Input: part model. Units: mm. Frame: model coordinates. Face numbers are marked on the shaded views. A direction names the side the tool comes from. Give positions to 0.01 mm unless a question says otherwise; leave off trailing zeros. Write each loop counter-clockwise with the first axis right and the second up, starting at its lowest first coordinate (ties: lowest second). Pieces come first, ordered by that corner, then holes. Notation, with made-up numbers: (82, 61) - (89, 61) arc R14 ccw to (89, 83) - close; hole circle Ø10 at (6, 85.25). An arc over 180 degrees is marked (long way). Use a Markdown table: item, result. Add a question column.
1. Section query D-D, the plane y = 53. Return loops of the section in (x, z).
2. Section query B-B, the plane z = -82.5. Return loops of the section in (x, y), plus the area to 3 significant figures.
3. Section query C-C, the plane x = 6.5. Return loops of the section in (y, z).
4. Set-up query: the marked faces 1, 2, 3, 4 and 5. Return all of +Z, -Z, +X, -X, +Y, -Y with unobstructed straight access to the full face (end or side cutting, diameter ignored); none if empty.
5. Material intervals for probe 1 along X at (y, z) = (-10, -135); probe 2 along Z at (x, y) = (19, -50); probe 3 along X at (y, z) = (86, -74.5), sorted ascending.
6. Section query A-A, the plane x = 39. Return loops of the section in (y, z), plus the area to 3 significant figures.
7. Pin query (flat end, axial travel): pin 1 (12 mm diameter, centred on x = 1.5, z = -126, fed in from +Y); pin 2 (2 mm diameter, centred on x = -46.5, y = 85, fed in from -Z); pin 3 (4 mm diameter, centred on y = 72, z = -111, fed in from +X); pin 4 (5 mm diameter, centred on x = 6, y = -40.5, fed in from -Z). Return the tip coordinate at first contact, or that it passes through.
8. Mould query, pull axis X, two halves, no side actions, for the marked faces 6, 7 and 8. Classes: released by +X, released by -X, zero draft, split by the parting line, or undercut.
```python
from build123d import *

# Parameters (mm, degrees)
BASE_PLATE_SKETCH_R      = 10
BASE_PLATE_DEPTH         = 25
FLANGE_SKETCH_W          = 130
FLANGE_SKETCH_H          = 25
FLANGE_DEPTH             = 160
FLANGE_PROFILE_CUT_DEPTH = 160
HOLES_SKETCH_R           = 10
HOLES_CUT_DEPTH          = 160
LUG_SKETCH_R             = 15
LUG_DEPTH                = 136
LUG_45DEG_TRIM_DEPTH     = 136
LUG_NOTCH_DEPTH          = 136


with BuildPart() as part:
    # Base Plate Sketch → Base Plate (new body)
    with BuildSketch(Plane.XY):
        with BuildLine():
            Line((-69.89539749, 0), (60.10460251, 0))
            Line((60.10460251, 0), (60.10460251, -65))
            ThreePointArc((60.10460251, -65), (52.78227204, -82.67766953), (35.10460251, -90))
            Line((35.10460251, -90), (-44.89539749, -90))
            ThreePointArc((-44.89539749, -90), (-62.573067019, -82.67766953), (-69.89539749, -65))
            Line((-69.89539749, -65), (-69.89539749, 0))
        make_face()
        with Locations((-44.89539749, -65)):
            Circle(BASE_PLATE_SKETCH_R, mode=Mode.SUBTRACT)
        with Locations((35.10460251, -65)):
            Circle(BASE_PLATE_SKETCH_R, mode=Mode.SUBTRACT)
    extrude(amount=BASE_PLATE_DEPTH)

    # Flange Sketch → Flange (add)
    with BuildSketch(Plane(origin=(0, 0, 0), x_dir=(-1, 0, 0), z_dir=(0, 0, -1))):
        with Locations((4.89539749, -12.5)):
            Rectangle(FLANGE_SKETCH_W, FLANGE_SKETCH_H)
    extrude(amount=FLANGE_DEPTH)

    # Flange Profile Cut Sketch → Flange Profile Cut (cut)
    with BuildSketch(Plane(origin=(0, 0, 0), x_dir=(1, 0, 0), z_dir=(0, 1, 0))):
        with BuildLine():
            Line((60.10460251, 160), (35.10460251, 160))
            ThreePointArc((35.10460251, 160), (52.78227204, 152.67766953), (60.10460251, 135))
            Line((60.10460251, 135), (60.10460251, 160))
        make_face()
        with BuildLine():
            ThreePointArc((-69.89539749, 135), (-62.573067019, 152.67766953), (-44.89539749, 160))
            Line((-44.89539749, 160), (-69.89539749, 160))
            Line((-69.89539749, 160), (-69.89539749, 135))
        make_face()
    extrude(amount=-FLANGE_PROFILE_CUT_DEPTH, mode=Mode.SUBTRACT)

    # Holes Sketch → Holes Cut (cut)
    with BuildSketch(Plane(origin=(0, 0, 0), x_dir=(1, 0, 0), z_dir=(0, 1, 0))):
        with Locations(Location((-44.89539749, 135, 0), (0, 0, 270))):
            Circle(HOLES_SKETCH_R)
        with Locations(Location((35.10460251, 135, 0), (0, 0, 270))):
            Circle(HOLES_SKETCH_R)
    extrude(amount=-HOLES_CUT_DEPTH, mode=Mode.SUBTRACT)

    # Lug Sketch → Lug (add)
    with BuildSketch(Plane(origin=(0, 0, 0), x_dir=(1, 0, 0), z_dir=(0, 1, 0))):
        with BuildLine():
            Line((-44.89539749, -25), (35.10460251, -25))
            Line((35.10460251, -25), (35.10460251, 75))
            ThreePointArc((35.10460251, 75), (-4.89539749, 115), (-44.89539749, 75))
            Line((-44.89539749, 75), (-44.89539749, -25))
        make_face()
        with Locations(Location((-4.89539749, 75, 0), (0, 0, 270))):
            Circle(LUG_SKETCH_R, mode=Mode.SUBTRACT)
    extrude(amount=LUG_DEPTH)

    # Lug 45deg Trim Sketch → Lug 45deg Trim (cut)
    with BuildSketch(Plane(origin=(35.10460251, 0, 0), x_dir=(0, 0, -1), z_dir=(1, 0, 0))):
        Polygon((-25, 0), (-25, 136), (115, 136), align=None)
    extrude(amount=-LUG_45DEG_TRIM_DEPTH, mode=Mode.SUBTRACT)

    # Lug Notch Sketch → Lug Notch (cut)
    with BuildSketch(Plane(origin=(35.10460251, 0, 0), x_dir=(0, 0, -1), z_dir=(1, 0, 0))):
        Polygon((-7.068015479, 17.419642107), (3.691175234, 27.871427371), (14.142960498, 17.112236658), (3.383769785, 6.660451394), align=None)
    extrude(amount=-LUG_NOTCH_DEPTH, mode=Mode.SUBTRACT)


solid = part.part
```
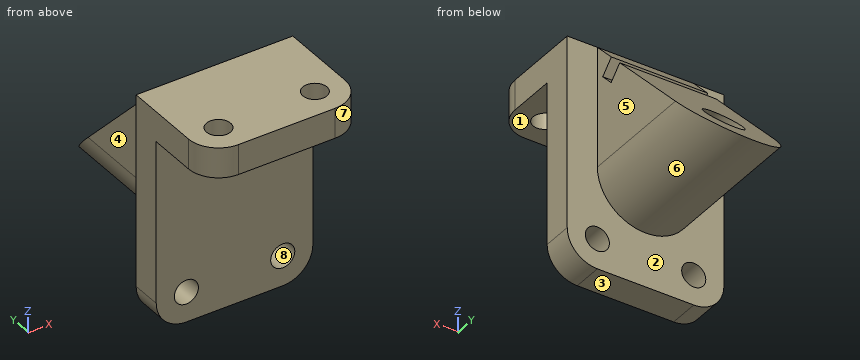
Result sheet:
| question | item | result |
|---|---|---|
| 1 | outline | (-44.9, -75) arc R40 ccw to (35.1, -75) - (35.1, -29.56) - (-44.9, -29.56) - close; hole circle Ø30 at (-4.9, -75) |
| 2 | outline | (-69.9, -25) - (60.1, -25) - (60.1, 0) - (34.4, 0) - (34.4, 104.43) - (8.09, 104.43) - (8.09, 0) - (-17.89, 0) - (-17.89, 104.43) - (-44.19, 104.43) - (-44.19, 0) - (-69.9, 0) - close |
| 2 | area | 8,740 mm² |
| 3 | outline | (-90, 0) - (-25, 0) - (-25, -160) - (0, -160) - (0, -113.34) - (134.39, -113.34) - (106.62, -84.75) - (0, -84.75) - (0, -65.25) - (87.67, -65.25) - (27.87, -3.69) - (17.11, -14.14) - (6.66, -3.38) - (17.42, 7.07) - (0, 25) - (-90, 25) - close |
| 4 | face 1 | -Z, +X, -X, -Y |
| 4 | face 2 | -Z, +Y |
| 4 | face 3 | -Z, +X, -X, +Y, -Y |
| 4 | face 4 | +Z, -Z, -X, +Y |
| 4 | face 5 | +Z, -Z, +X, +Y |
| 5 | probe 1 | x = -69.9 to -54.9, -34.9 to 25.1, 45.1 to 60.1 |
| 5 | probe 2 | z = 0 to 25 |
| 5 | probe 3 | x = -44.9 to -19.89, 10.1 to 35.1 |
| 6 | outline | (-89.69, 0) - (-74.21, 0) - (-74.21, 25) - (-89.69, 25) - close; (-55.79, 0) - (-25, 0) - (-25, -125.79) - (0, -125.79) - (0, 25) - (-55.79, 25) - close; (-25, -159.69) - (0, -159.69) - (0, -144.21) - (-25, -144.21) - close |
| 6 | area | 5,310 mm² |
| 7 | pin 1 | stops at y = 0 |
| 7 | pin 2 | passes through |
| 7 | pin 3 | stops at x = 16.18 |
| 7 | pin 4 | stops at z = 0 |
| 8 | face 6 | split by the parting line |
| 8 | face 7 | released by +X |
| 8 | face 8 | undercut |
